Could you check a few things on this model? Use its own coordinates, in mm. Face numbers are marked on the shaded views. A direction names the side the tool comes from. Round coordinates to 2 decimals unless told otherwise and drop trailing zeros. Order: outer loops, then holes, each group sorted by start corner. A loop starts at its lowest first (then second) coordinate and runs counter-clockwise, first axis right, second up. Notation, with made-up numbers: (12, -14) - (24, -14) arc R6 cw to (24, -5) - close; hole circle Ø1 at (-18, -16.75). An arc over 180 degrees is marked (long way). Use one line per item in the form item = value.
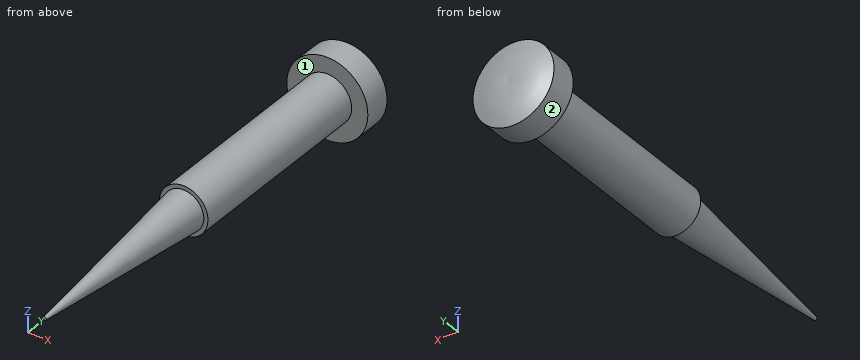
from build123d import *

# Parameters (mm, degrees)
TIP_BASE_CIRCLE_3_R      = 1.5
TAPERED_NEEDLE_TIP_DEPTH = 14.5
TAPERED_NEEDLE_TIP_TAPER = 5.42


with BuildPart() as part:
    # Head and Stem Profile → Head and Stem Revolve (revolve)
    with BuildSketch(Plane.XY, mode=Mode.PRIVATE) as head_and_stem_revolve_sk:
        with BuildLine():
            Line((0, 0), (0, 17.5))
            ThreePointArc((0, 17.5), (1.532206849, 17.443241097), (3, 17))
            Line((3, 17), (3, 15))
            Line((3, 15), (1.8, 15))
            Line((1.8, 15), (1.8, 0))
            Line((1.8, 0), (0, 0))
        make_face()
    revolve(head_and_stem_revolve_sk.sketch.rotate(Axis((0, 0, 0), (0, 1, 0)), 90), axis=Axis((0, 0, 0), (0, 1, 0)))

    # Tip Base Circle Ø3 → Tapered Needle Tip (add)
    with BuildSketch(Plane.XZ):
        Circle(TIP_BASE_CIRCLE_3_R)
    extrude(amount=TAPERED_NEEDLE_TIP_DEPTH, taper=TAPERED_NEEDLE_TIP_TAPER)


solid = part.part
Item 1: Imagine slicing it at B-B on y = -9. Please give me the cut outline in (x, z).
Found:
outline = circle Ø1.29 at (0, 0)
Item 2: Will these pins go through, and if not, where does the flat tip stop? P1, Ø1.5, axis at y = -1, z = 1.5, coming from the -X side; P2, Ø2, axis at x = 2, z = 0.5, coming from the +Y side; P3, Ø2, axis at y = 13, z = 0, coming from the -X side.
Found:
P1 = -1.2
P2 = 17.5
P3 = -1.8
Item 3: For the marked faces 1 and 2, which set-ups out of +Z, -Z, +X, -X, +Y, -Y let a thin tool reach every point of the face, with its end or its side?
Found:
face_1 = -Y
face_2 = +Y, -Y
Item 4: I need wall thicknesses on L1, parallel to Z at x = 0, y = -13; L2, parallel to Z at x = -0.75, y = -5.5; L3, parallel to Y at x = -1.75, z = 2. Which ranges of each line are inside material? Lowest first, please.
Found:
L1 = -0.27 to 0.27
L2 = -0.63 to 0.63
L3 = 15 to 17.14
Item 5: Imagine slicing it at A-A on y = 13. Please give me the cut outline in (x, z), plus the area to 3 significant figures.
Found:
outline = circle Ø3.6 at (0, 0)
area = 10.2 mm2
